Drawing for the job (mm, zero at the part's lowest x, y, z). A direction names the side the tool comes from. Coordinates: 2 decimals unless noted, no trailing zeros. Loops run counter-clockwise (first coordinate to the right, second up) from the corner with the lowest first, then second, coordinate; pieces in that order, holes last. Notation, with made-up numbers: (1, 73) - (52, 73) arc R23 cw to (52, 88) - close; hole circle Ø3 at (61, 27). An arc over 180 degrees is marked (long way). Put each result on its own line as item: value.
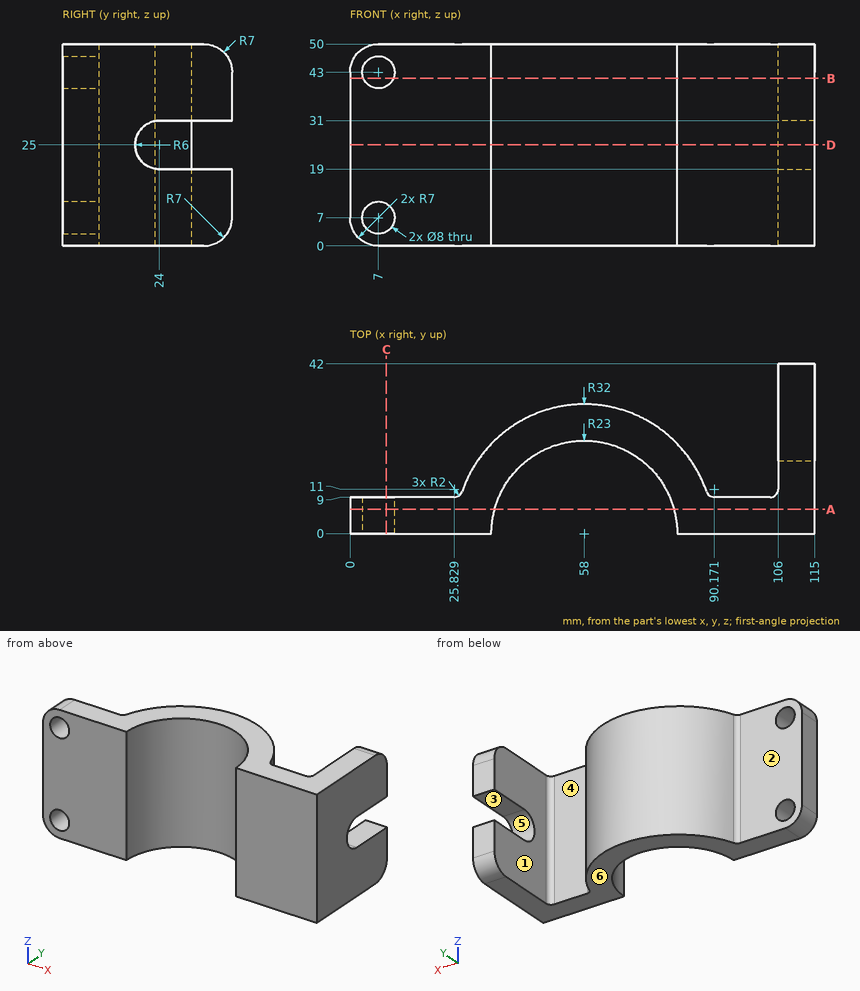
Q1. Pin check, flat tips, straight feed: pin 1 Ø10.5 at (x, z) = (7, 43) entering from +Y; pin 2 Ø2 at (y, z) = (34.5, 9) entering from -X; pin 3 Ø3 at (y, z) = (16.5, 36.5) entering from -X. Stop position of each tip, or through.
Determined:
pin 1: y = 9
pin 2: x = 106
pin 3: x = 29.73
Q2. Mould opens along Z. For the marked faces 4, 5 and 6 say: +Z half, -Z half, draft (parallel to the pull), parting line (faces both ways), or undercut.
Determined:
face 4: draft
face 5: undercut
face 6: -Z half
Q3. Wall check: L1, parallel to Z at x = 7, y = 7.25; L2, parallel to X at y = 2, z = 4.5 (1 decimal); L3, parallel to X at y = 35, z = 37.5. Give the ranges that are in metal, low to high. Write a range as from..to.
Determined:
L1: 0..3, 11..39, 47..50
L2: 0.5..3.9, 10.1..35.1, 80.9..115
L3: 106..115
Q4. Tool access for the marked faces 1, 2 and 3: list every direction of +Z, -Z, +X, -X, +Y, -Y with a clear straight run to the whole face (end or side of a thin tool).
Determined:
face 1: +Z, -Z, +Y
face 2: +Z, -Z, -X, +Y
face 3: +X, +Y
Q5. Slice it at A-A, the plane y = 6. Give the cut face in (x, z).
Determined:
outline: (0, 7) arc R7 ccw to (7, 0) - (35.8, 0) - (35.8, 50) - (7, 50) arc R7 ccw to (0, 43) - close; (80.2, 0) - (115, 0) - (115, 50) - (80.2, 50) - close; hole circle Ø8 at (7, 7); hole circle Ø8 at (7, 43)
Q6. Slice it at D-D, the plane z = 25. Give the cut face in (x, y).
Determined:
outline: (0, 0) - (35, 0) arc R23 cw to (81, 0) - (115, 0) - (115, 18) - (106, 18) - (106, 11) arc R2 cw to (104, 9) - (90.17, 9) arc R2 cw to (88.28, 10.35) arc R32 ccw to (27.72, 10.35) arc R2 cw to (25.83, 9) - (0, 9) - close
Q7. Slice it at C-C, the plane x = 9. Give the cut face in (y, z), then the cut area to 3 significant figures.
Determined:
outline: (0, 0) - (9, 0) - (9, 3.54) - (0, 3.54) - close; (0, 10.46) - (9, 10.46) - (9, 39.54) - (0, 39.54) - close; (0, 46.46) - (9, 46.46) - (9, 50) - (0, 50) - close
area: 325 mm2
Q8. Slice it at B-B, the plane z = 41.5. Give the cut face in (x, y).
Determined:
outline: (0, 0) - (3.29, 0) - (3.29, 9) - (0, 9) - close; (10.71, 0) - (35, 0) arc R23 cw to (81, 0) - (115, 0) - (115, 42) - (106, 42) - (106, 11) arc R2 cw to (104, 9) - (90.17, 9) arc R2 cw to (88.28, 10.35) arc R32 ccw to (27.72, 10.35) arc R2 cw to (25.83, 9) - (10.71, 9) - close
